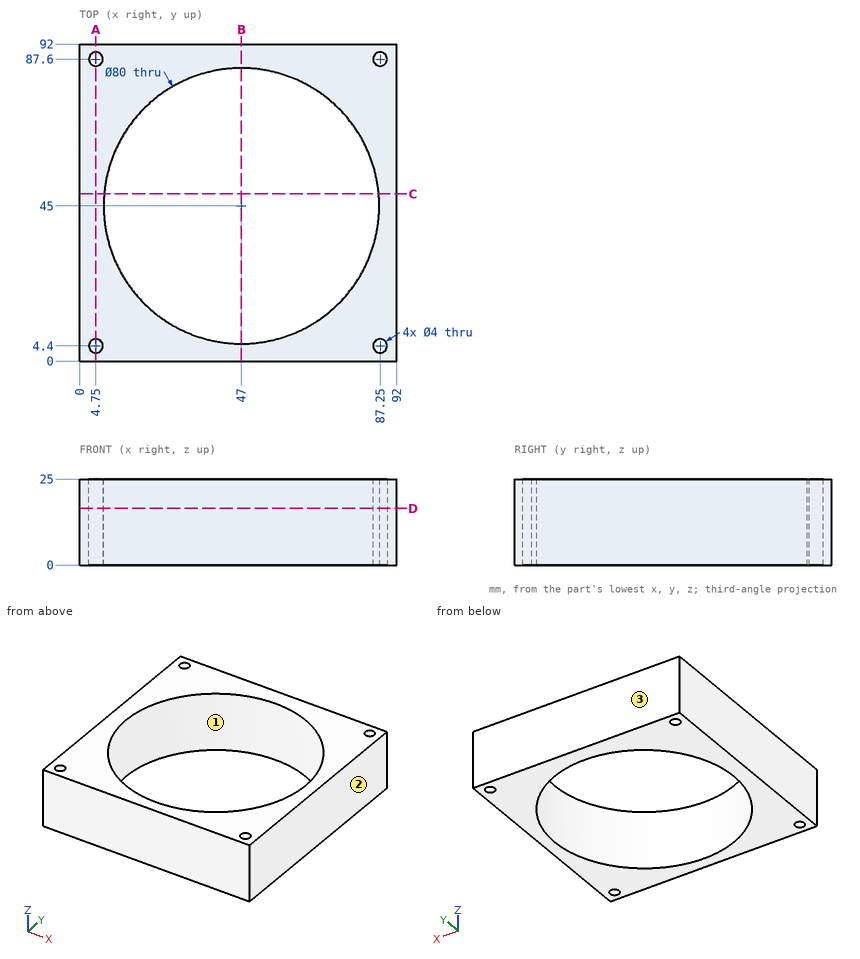
Design review of the part shown in the three views and the two pictorial views. Dimensions are in mm from the part's minimum x, y and z. Give positions to 0.01 mm unless a question says otherwise; leave off trailing zeros. Order: outer loops, then holes, each group sorted by start corner. A loop starts at its lowest first (then second) coordinate and runs counter-clockwise, first axis right, second up. Notation, with made-up numbers: M 0.5,26 L 42.5,26 A10 cw 42.5,44 Z; hole C -35,-33 d6. An arc over 180 degrees is marked long. Answer in a Markdown table with one row per item. Add a question column.
(1) For pin 1 (2.5 mm diameter, centred on x = 4.75, y = 4.4, fed in from +Z), flat-tipped, find the tip position at first contact; note if it passes through.
(2) Mouldability with a two-part tool opening along Y and no side actions: class the marked faces 1, 2 and 3 as +Y half, -Y half, draft (parallel to the pull), parting line (faces both ways), or undercut.
(3) Consider section A-A on x = 4.75. State the section outline as (y, z) points.
(4) Consider section D-D on z = 16.5. State the section outline as (x, y) points.
(5) Consider section C-C on y = 48.5. State the section outline as (x, z) points, and give its area (3 significant figures).
(6) Consider section B-B on x = 47. State the section outline as (y, z) points.
(7) Wall thickness on probe 1 along Y at (x, z) = (4.75, 18); probe 2 along Y at (x, z) = (47, 13); probe 3 along X at (y, z) = (54, 22.5): over which ranges is each line inside the solid? List them lowest first. Write a range as [from, to].
Evaluation:
| question | item | result |
|---|---|---|
| 1 | pin 1 | passes through |
| 2 | face 1 | undercut |
| 2 | face 2 | draft |
| 2 | face 3 | +Y half |
| 3 | outline | M 0,0 L 2.4,0 L 2.4,25 L 0,25 Z; M 6.4,0 L 85.6,0 L 85.6,25 L 6.4,25 Z; M 89.6,0 L 92,0 L 92,25 L 89.6,25 Z |
| 4 | outline | M 0,0 L 92,0 L 92,92 L 0,92 Z; hole C 4.75,4.4 d4; hole C 4.75,87.6 d4; hole C 47,45 d80; hole C 87.25,4.4 d4; hole C 87.25,87.6 d4 |
| 5 | outline | M 0,0 L 7.15,0 L 7.15,25 L 0,25 Z; M 86.85,0 L 92,0 L 92,25 L 86.85,25 Z |
| 5 | area | 308 mm^2 |
| 6 | outline | M 0,0 L 5,0 L 5,25 L 0,25 Z; M 85,0 L 92,0 L 92,25 L 85,25 Z |
| 7 | probe 1 | y = [0, 2.4], [6.4, 85.6], [89.6, 92] |
| 7 | probe 2 | y = [0, 5], [85, 92] |
| 7 | probe 3 | x = [0, 8.03], [85.97, 92] |
